```python
from build123d import *

# Parameters (mm, degrees)
SKETCH1_W                                            = 60
SKETCH1_H                                            = 80
BOSS_EXTRUDE1_DEPTH                                  = 12
M4_TAPPED_HOLE1_D                                    = 3.3
CBORE_FOR_M4_HEXAGON_SOCKET_HEAD_CAP_SCR_D           = 4.5
CBORE_FOR_M4_HEXAGON_SOCKET_HEAD_CAP_SCR_CBORE_D     = 8
CBORE_FOR_M4_HEXAGON_SOCKET_HEAD_CAP_SCR_CBORE_DEPTH = 4.6
CHAMFER1_SIZE                                        = 1


with BuildPart() as part:
    # Sketch1 → Boss-Extrude1 (new body)
    with BuildSketch(Plane(origin=(0, 0, 0), x_dir=(0, 0, -1), z_dir=(1, 0, 0))):
        Rectangle(SKETCH1_W, SKETCH1_H)
    extrude(amount=BOSS_EXTRUDE1_DEPTH)

    # M4 Tapped Hole1 (through all)
    with Locations(Plane.ZY):
        with Locations((-25, 27.5), (-25, -22.5), (25, -22.5), (25, 27.5)):
            Hole(M4_TAPPED_HOLE1_D / 2)

    # CBORE for M4 Hexagon socket head cap screws1 (through all)
    with Locations(Plane.ZY):
        with Locations((0, -25), (0, 25)):
            CounterBoreHole(CBORE_FOR_M4_HEXAGON_SOCKET_HEAD_CAP_SCR_D / 2, CBORE_FOR_M4_HEXAGON_SOCKET_HEAD_CAP_SCR_CBORE_D / 2, CBORE_FOR_M4_HEXAGON_SOCKET_HEAD_CAP_SCR_CBORE_DEPTH)

    # Chamfer1
    chamfer1_edges = [part.edges().sort_by_distance(p)[0] for p in [
        (6, -40, -30),
        (6, -40, 30),
        (6, 40, 30),
        (6, 40, -30),
    ]]
    chamfer(chamfer1_edges, length=CHAMFER1_SIZE)


solid = part.part
```
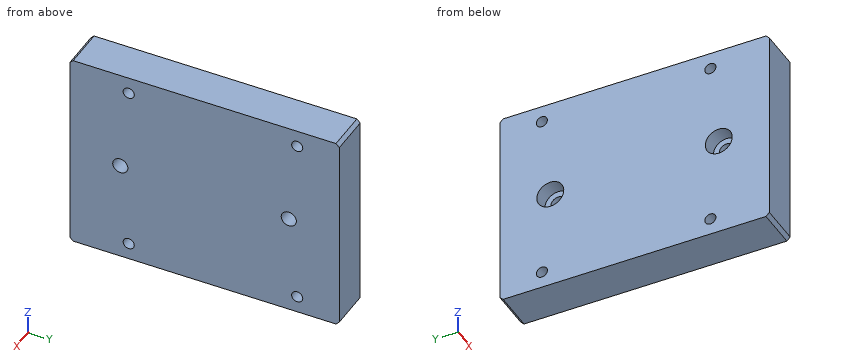
For this review, take the finished solid that the model builds, in its own axes (mm). Coordinates: 2 decimals unless noted, no trailing zeros. Write each loop counter-clockwise with the first axis right and the second up, starting at its lowest first coordinate (ties: lowest second). Pieces come first, ordered by that corner, then holes.
(1) Add section A-A on z = -25. Give the boundary of the cut face in (x, y), then the cut area to 3 significant figures.
(2) Wall thickness on probe 1 along Y at (x, z) = (2.9, 0); probe 2 along Z at (x, y) = (3, 27); probe 3 along X at (y, z) = (22, -2.5): over which ranges is each line inside the solid? List them lowest first.
(3) Add section B-B on y = -25. Give the boundary of the cut face in (x, z).
(4) For pin 1 Ø4 at (y, z) = (25, 0) entering from -X; pin 2 Ø6.5 at (y, z) = (-25, 0) entering from -X, all flat-tipped, find the tip position at first contact; note any pin that passes through.
Answer sheet:
1. outline: (0, -40) - (12, -40) - (12, -24.15) - (0, -24.15) - close; (0, -20.85) - (12, -20.85) - (12, 25.85) - (0, 25.85) - close; (0, 29.15) - (12, 29.15) - (12, 40) - (0, 40) - close
1. area: 881 mm2
2. probe 1: y = -40 to -29, -21 to 21, 29 to 40
2. probe 2: z = -30 to -26.57, -23.43 to -3.46, 3.46 to 23.43, 26.57 to 30
2. probe 3: x = 4.6 to 12
3. outline: (0, -30) - (12, -30) - (12, -2.25) - (4.6, -2.25) - (4.6, -4) - (0, -4) - close; (0, 4) - (4.6, 4) - (4.6, 2.25) - (12, 2.25) - (12, 30) - (0, 30) - close
4. pin 1: passes through
4. pin 2: stops at x = 4.6
